```python
from build123d import *

# Parameters (mm, degrees)
SKETCH1_R           = 5
SKETCH1_R_2         = 2.6
BOSS_EXTRUDE1_DEPTH = 5


with BuildPart() as part:
    # Sketch1 → Boss-Extrude1 (new body)
    with BuildSketch(Plane.XY):
        with BuildLine():
            Line((-7.412562463, -1.141892169), (-0.198568318, -47.971342146))
            ThreePointArc((-0.198568318, -47.971342146), (4.453004984, -53.802751838), (11.835747448, -52.736174654))
            Line((11.835747448, -52.736174654), (63.035902792, -12.674296032))
            ThreePointArc((63.035902792, -12.674296032), (65.633751361, -4.735983598), (59.277288615, 0.682595814))
            Line((59.277288615, 0.682595814), (0.863139126, 7.450167169))
            ThreePointArc((0.863139126, 7.450167169), (-5.401815198, 5.202921542), (-7.412562463, -1.141892169))
        make_face()
        with Locations((58.414149489, -6.767571355)):
            Circle(SKETCH1_R, mode=Mode.SUBTRACT)
        with Locations((7.213994146, -46.829449977)):
            Circle(SKETCH1_R_2, mode=Mode.SUBTRACT)
        Circle(SKETCH1_R_2, mode=Mode.SUBTRACT)
        with BuildLine():
            Line((38.716618419, -7.505580332), (10.080053588, -4.187891081))
            ThreePointArc((10.080053588, -4.187891081), (5.903417372, -5.686054833), (4.562919195, -9.91593064))
            Line((4.562919195, -9.91593064), (8.099459791, -32.873289294))
            ThreePointArc((8.099459791, -32.873289294), (11.200508659, -36.760895756), (16.122336968, -36.049844299))
            Line((16.122336968, -36.049844299), (41.222361204, -16.410174896))
            ThreePointArc((41.222361204, -16.410174896), (42.95426025, -11.117966607), (38.716618419, -7.505580332))
        make_face(mode=Mode.SUBTRACT)
    extrude(amount=BOSS_EXTRUDE1_DEPTH)


solid = part.part
```
Verification items for the finished model (mm, model axes). A direction names the side the tool comes from. Coordinates: 2 decimals unless noted, no trailing zeros. Loops run counter-clockwise (first coordinate to the right, second up) from the corner with the lowest first, then second, coordinate; pieces in that order, holes last. Notation, with made-up numbers: (63, 27.25) -> (107, 27.25) arc R21 ccw to (107, 56.25) -> close; hole circle Ø8 at (-16, 3.5). An arc over 180 degrees is marked (long way). Answer in a Markdown table with one row per item.
1) Depth check by flat-ended pin: P1, Ø8, axis at x = 20, y = -11.5, coming from the +Z side; P2, Ø2, axis at x = 26.5, z = 1, coming from the -Y side. Enter the tip coordinate at first touch or a pass-through.
The answers:
| item | result |
|---|---|
| P1 | passes through |
| P2 | stops at y = -42.04 |
2) Section check D-D (x = 17). Record the cut outline in (y, z), and give its area (3 significant figures).
The answers:
| item | result |
|---|---|
| outline | (-48.7, 0) -> (-35.36, 0) -> (-35.36, 5) -> (-48.7, 5) -> close; (-4.99, 0) -> (5.58, 0) -> (5.58, 5) -> (-4.99, 5) -> close |
| area | 120 mm2 |
3) Section check A-A (y = -46). Record the cut outline in (x, z).
The answers:
| item | result |
|---|---|
| outline | (-0.5, 0) -> (4.75, 0) -> (4.75, 5) -> (-0.5, 5) -> close; (9.68, 0) -> (20.44, 0) -> (20.44, 5) -> (9.68, 5) -> close |
4) Access from +Z, -Z, +X, -X, +Y, -Y to the whole of each face (thin tool, end or side, straight path). Record for faces 1 (the face through (37.077, -32.986, 2.465)), 2 (the face through (24.6, -5.87, 2.46)).
The answers:
| item | result |
|---|---|
| face 1 | +Z, -Z, +X, -Y |
| face 2 | +Z, -Z |
5) Section check B-B (x = 7). Record the cut outline in (y, z), and give its area (3 significant figures).
The answers:
| item | result |
|---|---|
| outline | (-54.33, 0) -> (-49.42, 0) -> (-49.42, 5) -> (-54.33, 5) -> close; (-44.24, 0) -> (-25.74, 0) -> (-25.74, 5) -> (-44.24, 5) -> close; (-4.83, 0) -> (6.74, 0) -> (6.74, 5) -> (-4.83, 5) -> close |
| area | 175 mm2 |
6) Section check C-C (z = 3.4). Record the cut outline in (x, y).
The answers:
| item | result |
|---|---|
| outline | (-7.41, -1.14) -> (-0.2, -47.97) arc R7.5 ccw to (11.84, -52.74) -> (63.04, -12.67) arc R7.5 ccw to (59.28, 0.68) -> (0.86, 7.45) arc R7.5 ccw to start; hole circle Ø5.2 at (0, 0); hole (4.56, -9.92) -> (8.1, -32.87) arc R5 ccw to (16.12, -36.05) -> (41.22, -16.41) arc R5 ccw to (38.72, -7.51) -> (10.08, -4.19) arc R5 ccw to start; hole circle Ø5.2 at (7.21, -46.83); hole circle Ø10 at (58.41, -6.77) |
7) Draft check along Y on faces 3 (the face through (30.48, 4.02, 2.46)), 4 (the face through (6.3, -21.2, 2.5)), 5 (the face through (65.666, -4.856, 2.465)), 6 (the face through (29, -30, 0)). Enter one of: released by +Y, released by -Y, zero draft, split by the parting line, or undercut.
The answers:
| item | result |
|---|---|
| face 3 | released by +Y |
| face 4 | undercut |
| face 5 | split by the parting line |
| face 6 | zero draft |
8) Scan lines: line 1 along Y through (x, z) = (9, 3.9); line 2 along X through (y, z) = (-9, 1); line 3 along X through (y, z) = (-10.5, 0.6). Record each from-to range of solid material in increasing order. Write a range as from..to.
The answers:
| item | result |
|---|---|
| line 1 | y = -54.11..-48.72, -44.94..-35.06, -4.18..6.51 |
| line 2 | x = -6.2..4.51, 41.74..53.94, 62.89..65.57 |
| line 3 | x = -5.97..4.65, 42.74..55.09, 61.74..64.92 |
